```python
from build123d import *

# Parameters (mm, degrees)
SKETCH1_W          = 14
SKETCH1_H          = 20
BOSS_EXTRUDE_DEPTH = 8
SKETCH2_R          = 5
CUT_EXTRUDE1_DEPTH = 3.5
SKETCH3_R          = 2.75
CUT_EXTRUDE2_DEPTH = 25.824383175
CHAMFER1_SIZE      = 1


with BuildPart() as part:
    # Sketch1 → Boss-Extrude (new body)
    with BuildSketch(Plane.XY):
        with Locations((-7, 10)):
            Rectangle(SKETCH1_W, SKETCH1_H)
    extrude(amount=-BOSS_EXTRUDE_DEPTH)

    # Sketch2 → Cut-Extrude1 (cut)
    with BuildSketch(Plane.XY):
        with Locations((-7, 10)):
            Circle(SKETCH2_R)
    extrude(amount=-CUT_EXTRUDE1_DEPTH, mode=Mode.SUBTRACT)

    # Sketch3 → Cut-Extrude2 (cut, through all)
    with BuildSketch(Plane.XY.offset(-3.5)):
        with Locations((-7, 10)):
            Circle(SKETCH3_R)
    extrude(amount=-CUT_EXTRUDE2_DEPTH, mode=Mode.SUBTRACT)

    # Chamfer1
    chamfer1_edges = [part.edges().sort_by_distance(p)[0] for p in [
        (-14, 10, -8),
        (0, 10, -8),
        (-14, 10, 0),
        (0, 10, 0),
    ]]
    chamfer(chamfer1_edges, length=CHAMFER1_SIZE)


solid = part.part
```
Input: part model. Units: mm. Frame: model coordinates. A direction names the side the tool comes from. Round coordinates to 2 decimals unless told otherwise and drop trailing zeros. Loops run counter-clockwise (first coordinate to the right, second up) from the corner with the lowest first, then second, coordinate; pieces in that order, holes last. Notation, with made-up numbers: (45.25, -13.5) -> (64.25, -13.5) arc R14 ccw to (64.25, 8.5) -> close; hole circle Ø6 at (56, 19). An arc over 180 degrees is marked (long way). One line per item, written item: value.
(1) Material intervals for line 1 (Y direction, x = -7, z = -4.95); line 2 (Y direction, x = -7, z = -3.25); line 3 (Z direction, x = -10.25, y = 9.5), sorted ascending. Write a range as [from, to].
Geometry check:
line 1: [0, 7.25], [12.75, 20]
line 2: [0, 5], [15, 20]
line 3: [-8, -3.5]
(2) Section A-A (x = -7). Return the cut outline in (y, z).
Geometry check:
outline: (0, -8) -> (7.25, -8) -> (7.25, -3.5) -> (5, -3.5) -> (5, 0) -> (0, 0) -> close; (12.75, -8) -> (20, -8) -> (20, 0) -> (15, 0) -> (15, -3.5) -> (12.75, -3.5) -> close
(3) Set-up query: faces 4 (the face through (-4.8, 7.8, -3.5)), 5 (the face through (-14, 10, -4)). Return all of +Z, -Z, +X, -X, +Y, -Y with unobstructed straight access to the full face (end or side cutting, diameter ignored); none if empty.
Geometry check:
face 4: +Z
face 5: +Z, -Z, -X, +Y, -Y
(4) Section B-B (y = 10). Return the cut outline in (x, z), plus the area to 4 significant figures.
Geometry check:
outline: (-14, -7) -> (-13, -8) -> (-9.75, -8) -> (-9.75, -3.5) -> (-12, -3.5) -> (-12, 0) -> (-13, 0) -> (-14, -1) -> close; (-4.25, -8) -> (-1, -8) -> (0, -7) -> (0, -1) -> (-1, 0) -> (-2, 0) -> (-2, -3.5) -> (-4.25, -3.5) -> close
area: 50.25 mm2
(5) Section D-D (y = 16.25). Return the cut outline in (x, z).
Geometry check:
outline: (-14, -7) -> (-13, -8) -> (-1, -8) -> (0, -7) -> (0, -1) -> (-1, 0) -> (-13, 0) -> (-14, -1) -> close
(6) Mould query, pull axis Y, two halves, no side actions, for faces 1 (the face through (-2.23, 11.5, -1.73)), 2 (the face through (-7, 20, -4)), 3 (the face through (-0.5, 9.9, -7.5)). Classes: pulls with the +Y half, pulls with the -Y half, needs draft (parallel to the pull), parting line crosses it, or undercut.
Geometry check:
face 1: undercut
face 2: pulls with the +Y half
face 3: needs draft
(7) Section C-C (z = -0.75). Return the cut outline in (x, y), plus the area to 3 significant figures.
Geometry check:
outline: (-13.75, 0) -> (-0.25, 0) -> (-0.25, 20) -> (-13.75, 20) -> close; hole circle Ø10 at (-7, 10)
area: 191 mm2
(8) Pin query (flat end, axial travel): pin 1 (5 mm diameter, centred on x = -7, y = 10, fed in from -Z); pin 2 (3 mm diameter, centred on x = -9, y = 7.5, fed in from +Z); pin 3 (1.5 mm diameter, centred on x = -4.5, z = -1, fed in from -Y). Return the tip coordinate at first contact, or that it passes through.
Geometry check:
pin 1: through
pin 2: z = -3.5
pin 3: y = 0
